Here's how the part is built. I have some questions about the finished solid (model axes, mm). Face numbers are marked on the shaded views. A direction names the side the tool comes from. Coordinates: 2 decimals unless noted, no trailing zeros. Loops run counter-clockwise (first coordinate to the right, second up) from the corner with the lowest first, then second, coordinate; pieces in that order, holes last.
```python
from build123d import *

# Parameters (mm, degrees)
BOSS_EXTRUDE_1_DEPTH   = 15
SKETCH_4_R             = 3.25
CUT_EXTRUDE_1_DEPTH    = 74.654599313
LINEAR_PATTERN_1_COUNT = 2
LINEAR_PATTERN_1_PITCH = 15
SKETCH_5_R             = 3.25
CUT_EXTRUDE_2_DEPTH    = 91.691785736
LINEAR_PATTERN_2_COUNT = 2
LINEAR_PATTERN_2_PITCH = 15
CHAMFER_1_SIZE         = 2


with BuildPart() as part:
    # Sketch 3 → Boss-Extrude 1 (new body)
    with BuildSketch(Plane(origin=(0, 0, 0), x_dir=(1, 0, 0), z_dir=(0, 1, 0))):
        Polygon((40, 40), (20, 40), (20, 0), (0, -20), (-40, -20), (-40, -40), (40, -40), align=None)
    extrude(amount=BOSS_EXTRUDE_1_DEPTH)

    # Sketch 4 → Cut-Extrude 1 (cut, through all)
    with BuildSketch(Plane(origin=(0, 0, 20), x_dir=(-1, 0, 0), z_dir=(0, 0, -1))):
        with Locations((10, 7.5)):
            Circle(SKETCH_4_R)
    cut_extrude_1 = extrude(amount=-CUT_EXTRUDE_1_DEPTH, mode=Mode.SUBTRACT)

    # Linear Pattern 1: Cut-Extrude 1 ×2
    with Locations(*[(-i * LINEAR_PATTERN_1_PITCH, 0, 0) for i in range(1, LINEAR_PATTERN_1_COUNT)]):
        add(cut_extrude_1, mode=Mode.SUBTRACT)

    # Sketch 5 → Cut-Extrude 2 (cut, through all)
    with BuildSketch(Plane(origin=(40, 0, 0), x_dir=(0, 0, -1), z_dir=(1, 0, 0))):
        with Locations((10, 7.5)):
            Circle(SKETCH_5_R)
    cut_extrude_2 = extrude(amount=-CUT_EXTRUDE_2_DEPTH, mode=Mode.SUBTRACT)

    # Linear Pattern 2: Cut-Extrude 2 ×2
    with Locations(*[(0, 0, -i * LINEAR_PATTERN_2_PITCH) for i in range(1, LINEAR_PATTERN_2_COUNT)]):
        add(cut_extrude_2, mode=Mode.SUBTRACT)

    # Chamfer 1
    chamfer_1_edges = [part.edges().sort_by_distance(p)[0] for p in [
        (40, 7.5, 40),
    ]]
    chamfer(chamfer_1_edges, length=CHAMFER_1_SIZE)


solid = part.part
```
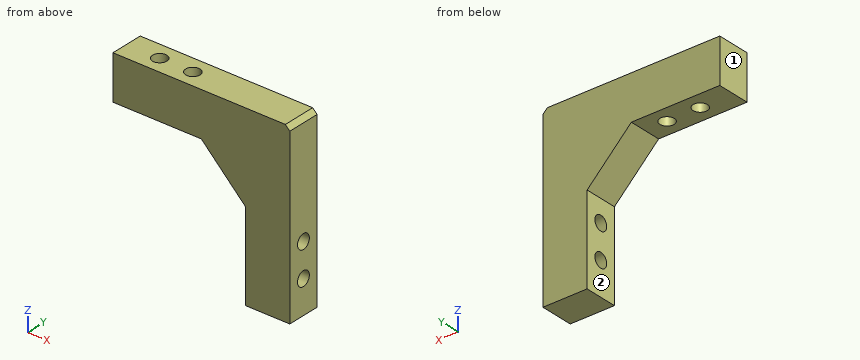
1. For pin 1 (6 mm diameter, centred on y = 11.5, z = -8, fed in from -X); pin 2 (5 mm diameter, centred on x = -5.5, z = 22.5, fed in from -Y); pin 3 (7.5 mm diameter, centred on x = -21, y = 5, fed in from -Z), each with a flat end and sliding along its axis, tell me the tip position at first contact or that it passes through.
2. I need wall thicknesses on line 1 along Y through (x, z) = (28, -10); line 2 along Z through (x, y) = (-3, 14.5). Which ranges of each line are inside material? Lowest first, please.
3. I want a section at B-B (x = -10). Please give me the cut outline in (y, z), then the cut area to 3 significant figures.
4. I want a section at C-C (z = -10). Please give me the cut outline in (x, y), then the cut area to 3 significant figures.
5. I want a section at D-D (x = 23). Please give me the cut outline in (y, z).
6. On a 3-axis mill with a long thin cutter (end or side, diameter ignored), from which of +Z, -Z, +X, -X, +Y, -Y can I reach the whole of each face in a straight line? I mean the marked faces 1 and 2. Say none if no direction works.
7. I want a section at A-A (y = 7.5). Please give me the cut outline in (x, z).
Response values:
1. pin 1: stops at x = 20
1. pin 2: stops at y = 0
1. pin 3: stops at z = 20
2. line 1: y = 0 to 4.25, 10.75 to 15
2. line 2: z = 20 to 40
3. outline: (0, 20) - (4.25, 20) - (4.25, 40) - (0, 40) - close; (10.75, 20) - (15, 20) - (15, 40) - (10.75, 40) - close
3. area: 170 mm2
4. outline: (20, 0) - (40, 0) - (40, 4.25) - (20, 4.25) - close; (20, 10.75) - (40, 10.75) - (40, 15) - (20, 15) - close
4. area: 170 mm2
5. outline: (0, -40) - (15, -40) - (15, 40) - (0, 40) - close; hole circle Ø6.5 at (7.5, -25); hole circle Ø6.5 at (7.5, -10)
6. face 1: +Z, -Z, -X, +Y, -Y
6. face 2: -Z, -X, +Y, -Y
7. outline: (-40, 20) - (-28.25, 20) - (-28.25, 40) - (-40, 40) - close; (-21.75, 20) - (-13.25, 20) - (-13.25, 40) - (-21.75, 40) - close; (-6.75, 20) - (0, 20) - (20, 0) - (20, -6.75) - (40, -6.75) - (40, 38) - (38, 40) - (-6.75, 40) - close; (20, -40) - (40, -40) - (40, -28.25) - (20, -28.25) - close; (20, -21.75) - (40, -21.75) - (40, -13.25) - (20, -13.25) - close
